Geometry: final body of the model. Coordinates: model frame, mm. A direction names the side the tool comes from. Round coordinates to 2 decimals unless told otherwise and drop trailing zeros. Loops run counter-clockwise (first coordinate to the right, second up) from the corner with the lowest first, then second, coordinate; pieces in that order, holes last. Notation, with made-up numbers: (61, 42) - (110, 42) arc R9 ccw to (110, 54) - close; hole circle Ø10 at (49, 71). An arc over 180 degrees is marked (long way). Answer as a JSON object with one key per item and string values. Group by question number.
Item 1: Section A-A (y = 0). Return the cut outline in (x, z).
Item 2: First-contact query: pin 1 (1 mm diameter, centred on x = 11, y = -13.5, fed in from -Z); pin 2 (8 mm diameter, centred on y = 5, z = 96.5, fed in from -X) (3 decimals); pin 3 (10 mm diameter, centred on y = -14, z = 130, fed in from -X); pin 4 (3 mm diameter, centred on x = 13.5, y = -7.5, fed in from -Z). Flat tips, straight axial feed; report the tip coordinate or a pass-through.
Item 3: Section B-B (z = 41). Return the cut outline in (x, y), plus the area to 3 significant figures.
Item 4: Line query: line 1 (Z direction, x = -0.5, y = -11.5); line 2 (Z direction, x = 0, y = 14.5); line 3 (Z direction, x = 4.5, y = -15). Output: solid intervals per line, ascending.
Item 5: Section D-D (z = 141.5). Return the cut outline in (x, y), plus the area to 3 significant figures.
Item 6: Section C-C (z = 81). Return the cut outline in (x, y), plus the area to 3 significant figures.
Item 7: Reachability of faces 4 (the face through (4, 13, 22)), 5 (the face through (0, -13, 65)), 6 (the face through (-3.794, -17.084, 151.44)), 7 (the face through (0, 15, 164)), 8 (the face through (-3.47, -15.62, 192.74)) from +Z, -Z, +X, -X, +Y, -Y: full face, straight path, thin tool, end or side. Return the list, or none.
Item 8: Draft query along Z for faces 1 (the face through (0, 0, 200)), 2 (the face through (-4.336, -19.524, 97.804)), 3 (the face through (0, -11, 57)). Return one class per face: released by +Z, released by -Z, zero draft, split by the parting line, or undercut.
```python
from build123d import *
from OCP.BRepFilletAPI import BRepFilletAPI_MakeChamfer

# Parameters (mm, degrees)
SKETCH1_R           = 15
BOSS_EXTRUDE1_DEPTH = 68
SKETCH2_R           = 17.5
BOSS_EXTRUDE2_DEPTH = 16
SKETCH3_R           = 20
BOSS_EXTRUDE3_DEPTH = 28
SKETCH4_R           = 17.5
BOSS_EXTRUDE4_DEPTH = 80
SKETCH5_R           = 16
BOSS_EXTRUDE5_DEPTH = 1.5
SKETCH6_R           = 17.5
BOSS_EXTRUDE6_DEPTH = 6.5
CUT_EXTRUDE1_START  = 17.5
CUT_EXTRUDE1_DEPTH  = 5
CUT_EXTRUDE2_START  = 15
CUT_EXTRUDE2_DEPTH  = 4
CUT_EXTRUDE3_START  = -15
CUT_EXTRUDE3_DEPTH  = 4
CHAMFER1_SIZE       = 0.5
CHAMFER1_SIZE2      = 0.288675135


with BuildPart() as part:
    # Sketch1 → Boss-Extrude1 (new body)
    with BuildSketch(Plane.XY):
        Circle(SKETCH1_R)
    extrude(amount=BOSS_EXTRUDE1_DEPTH)

    # Sketch2 → Boss-Extrude2 (add)
    with BuildSketch(Plane.XY.offset(68)):
        Circle(SKETCH2_R)
    extrude(amount=BOSS_EXTRUDE2_DEPTH)

    # Sketch3 → Boss-Extrude3 (add)
    with BuildSketch(Plane.XY.offset(84)):
        Circle(SKETCH3_R)
    extrude(amount=BOSS_EXTRUDE3_DEPTH)

    # Sketch4 → Boss-Extrude4 (add)
    with BuildSketch(Plane.XY.offset(112)):
        Circle(SKETCH4_R)
    extrude(amount=BOSS_EXTRUDE4_DEPTH)

    # Sketch5 → Boss-Extrude5 (add)
    with BuildSketch(Plane.XY.offset(192)):
        Circle(SKETCH5_R)
    extrude(amount=BOSS_EXTRUDE5_DEPTH)

    # Sketch6 → Boss-Extrude6 (add)
    with BuildSketch(Plane.XY.offset(193.5)):
        Circle(SKETCH6_R)
    extrude(amount=BOSS_EXTRUDE6_DEPTH)

    # Sketch7 → Cut-Extrude1 (cut)
    with BuildSketch(Plane(origin=(0, 0, 0), x_dir=(1, 0, 0), z_dir=(0, 1, 0)).offset(CUT_EXTRUDE1_START)):
        with BuildLine():
            Line((-5, -159), (-5, -121))
            ThreePointArc((-5, -121), (0, -116), (5, -121))
            Line((5, -121), (5, -159))
            ThreePointArc((5, -159), (0, -164), (-5, -159))
        make_face()
    extrude(amount=-CUT_EXTRUDE1_DEPTH, mode=Mode.SUBTRACT)

    # Sketch8 → Cut-Extrude2 (cut)
    with BuildSketch(Plane(origin=(0, 0, 0), x_dir=(1, 0, 0), z_dir=(0, 1, 0)).offset(CUT_EXTRUDE2_START)):
        with BuildLine():
            Line((-4, -44), (-4, 0))
            ThreePointArc((-4, 0), (0, 4), (4, 0))
            Line((4, 0), (4, -44))
            ThreePointArc((4, -44), (0, -48), (-4, -44))
        make_face()
    extrude(amount=-CUT_EXTRUDE2_DEPTH, mode=Mode.SUBTRACT)

    # Sketch9 → Cut-Extrude3 (cut)
    with BuildSketch(Plane(origin=(0, 0, 0), x_dir=(1, 0, 0), z_dir=(0, 1, 0)).offset(CUT_EXTRUDE3_START)):
        with BuildLine():
            Line((-4, -61), (-4, -54))
            ThreePointArc((-4, -54), (0, -50), (4, -54))
            Line((4, -54), (4, -61))
            ThreePointArc((4, -61), (0, -65), (-4, -61))
        make_face()
    extrude(amount=CUT_EXTRUDE3_DEPTH, mode=Mode.SUBTRACT)

    # Chamfer1: one chamfer whose edges measure the first distance from different faces: ONE call of the kernel's chamfer builder (chamfer() names one face for all edges)
    chamfer1_edges_1 = [part.edges().sort_by_distance(p)[0] for p in [
        (-17.5, 0, 200),
    ]]
    chamfer1_side_1 = [part.faces().sort_by_distance(p)[0] for p in [
        (-17.5, 0, 196.75),
    ]]
    chamfer1_edges_2 = [part.edges().sort_by_distance(p)[0] for p in [
        (-9.082951062, -11.937336386, 0),
    ]]
    chamfer1_side_2 = [part.faces().sort_by_distance(p)[0] for p in [
        (0, -0.583570782, 0),
    ]]
    chamfer1 = BRepFilletAPI_MakeChamfer(part.part.solid().wrapped)
    for e in chamfer1_edges_1:
        chamfer1.Add(CHAMFER1_SIZE, CHAMFER1_SIZE2, e.wrapped, chamfer1_side_1[0].wrapped)  # the first distance lies on this face
    for e in chamfer1_edges_2:
        chamfer1.Add(CHAMFER1_SIZE, CHAMFER1_SIZE2, e.wrapped, chamfer1_side_2[0].wrapped)  # the first distance lies on this face
    add(Compound.cast(chamfer1.Shape()), mode=Mode.REPLACE)


solid = part.part
```
Values:
{
 "1": {"outline": "(-20, 84) - (-17.5, 84) - (-17.5, 68) - (-15, 68) - (-15, 0.29) - (-14.5, 0) - (14.5, 0) - (15, 0.29) - (15, 68) - (17.5, 68) - (17.5, 84) - (20, 84) - (20, 112) - (17.5, 112) - (17.5, 192) - (16, 192) - (16, 193.5) - (17.5, 193.5) - (17.5, 199.5) - (17.21, 200) - (-17.21, 200) - (-17.5, 199.5) - (-17.5, 193.5) - (-16, 193.5) - (-16, 192) - (-17.5, 192) - (-17.5, 112) - (-20, 112) - close"},
 "2": {"pin 1": "stops at z = 68", "pin 2": "stops at x = -19.975", "pin 3": "stops at x = -15.01", "pin 4": "stops at z = 0"},
 "3": {"outline": "(-4, 11) - (-4, 14.46) arc R15 ccw (long way) to (4, 14.46) - (4, 11) - close", "area": "676 mm^2"},
 "4": {"line 1": "z = 0 to 50.03, 64.97 to 200", "line 2": "z = 48 to 116, 164 to 200", "line 3": "z = 68 to 200"},
 "5": {"outline": "(-5, 12.5) - (-5, 16.77) arc R17.5 ccw (long way) to (5, 16.77) - (5, 12.5) - close", "area": "915 mm^2"},
 "6": {"outline": "circle Ø35 at (0, 0)", "area": "962 mm^2"},
 "7": {"face 4": "-Z, +Y", "face 5": "-Y", "face 6": "+Z", "face 7": "+Y", "face 8": "none"},
 "8": {"face 1": "released by +Z", "face 2": "zero draft", "face 3": "undercut"}
}
